Build history of the part. All positions in model axes, mm. A direction names the side the tool comes from. Round coordinates to 2 decimals unless told otherwise and drop trailing zeros. Loops run counter-clockwise (first coordinate to the right, second up) from the corner with the lowest first, then second, coordinate; pieces in that order, holes last. Notation, with made-up numbers: (48, -39) - (64, -39) arc R16 ccw to (64, -21) - close; hole circle Ø7 at (1, -0.75). An arc over 180 degrees is marked (long way). Use a Markdown table: item, result.
from build123d import *

# Parameters (mm, degrees)
SKETCH1_W                   = 85
SKETCH1_H                   = 80
BOSS_EXTRUDE1_DEPTH         = 40
M8_TAPPED_HOLE1_D           = 6.8
M8_TAPPED_HOLE1_DEPTH       = 22.25
M8_TAPPED_HOLE1_CSINK_D     = 8.05
M8_TAPPED_HOLE1_CSINK_ANGLE = 90
M8_TAPPED_HOLE1_TIP         = 2.042926105
SKETCH5_W                   = 20
SKETCH5_H                   = 54.3
CUT_EXTRUDE1_DEPTH          = 1
CUT_EXTRUDE2_DEPTH          = 12


with BuildPart() as part:
    # Sketch1 → Boss-Extrude1 (new body)
    with BuildSketch(Plane(origin=(0, 0, 0), x_dir=(1, 0, 0), z_dir=(0, 1, 0))):
        Rectangle(SKETCH1_W, SKETCH1_H)
    extrude(amount=BOSS_EXTRUDE1_DEPTH)

    # M8 Tapped Hole1
    with Locations(Plane(origin=(0, 0, 0), x_dir=(-1, 0, 0), z_dir=(0, -1, 0))):
        with Locations((7.5, 28), (-22.5, 0), (7.5, -28), (32.5, 0)):
            CounterSinkHole(M8_TAPPED_HOLE1_D / 2, M8_TAPPED_HOLE1_CSINK_D / 2, depth=M8_TAPPED_HOLE1_DEPTH, counter_sink_angle=M8_TAPPED_HOLE1_CSINK_ANGLE)
            with Locations((0, 0, -(M8_TAPPED_HOLE1_DEPTH + M8_TAPPED_HOLE1_TIP / 2))):  # 118° drill point
                Cone(0, M8_TAPPED_HOLE1_D / 2, M8_TAPPED_HOLE1_TIP, mode=Mode.SUBTRACT)

    # Sketch5 → Cut-Extrude1 (cut)
    with BuildSketch(Plane(origin=(0, 40, 0), x_dir=(1, 0, 0), z_dir=(0, 1, 0))):
        with Locations((-7.5, 0)):
            Rectangle(SKETCH5_W, SKETCH5_H)
    extrude(amount=-CUT_EXTRUDE1_DEPTH, mode=Mode.SUBTRACT)

    # Sketch6 → Cut-Extrude2 (cut, symmetric)
    with BuildSketch(Plane.ZY.offset(7.5)):
        with BuildLine():
            Line((-8.2, 40), (8.2, 40))
            ThreePointArc((8.2, 40), (6.414845549, 34.892186713), (1.836644737, 32.008333333))
            ThreePointArc((1.836644737, 32.008333333), (1.264123473, 32.045632996), (0.806331836, 32.391463415))
            ThreePointArc((0.806331836, 32.391463415), (0, 32.8), (-0.806331836, 32.391463415))
            ThreePointArc((-0.806331836, 32.391463415), (-1.264123473, 32.045632996), (-1.836644737, 32.008333333))
            ThreePointArc((-1.836644737, 32.008333333), (-6.414845549, 34.892186713), (-8.2, 40))
        make_face()
    extrude(amount=CUT_EXTRUDE2_DEPTH, both=True, mode=Mode.SUBTRACT)


solid = part.part
Q1. Probe line 1 (Z direction, x = -7.5, y = 16.75); line 2 (X direction, y = 7, z = 28); line 3 (Z direction, x = -32.5, y = 7). List the from-to ranges inside material, lowest first.
Results found:
| item | result |
|---|---|
| line 1 | z = -40 to -31.4, -24.6 to 24.6, 31.4 to 40 |
| line 2 | x = -42.5 to -10.9, -4.1 to 42.5 |
| line 3 | z = -40 to -3.4, 3.4 to 40 |
Q2. Which spindle directions (+Z, -Z, +X, -X, +Y, -Y) get a long thin tool onto all of the face, cutting with end or side? Do faces 1 (the face through (-29.36, 11.59, 1.3)), 2 (the face through (42.5, 20, 1)), 3 (the face through (-7.7, 35, 6.5)). Say none if no direction does.
Results found:
| item | result |
|---|---|
| face 1 | -Y |
| face 2 | +Z, -Z, +X, +Y, -Y |
| face 3 | +Y |
Q3. Cut at B-B, the plane y = 35. List the corners of the cut face in (x, z), plus the area to 3 significant figures.
Results found:
| item | result |
|---|---|
| outline | (-42.5, -40) - (42.5, -40) - (42.5, 40) - (-42.5, 40) - close; hole (-19.5, -6.5) - (4.5, -6.5) - (4.5, 6.5) - (-19.5, 6.5) - close |
| area | 6,490 mm2 |
Q4. Drop a flat-ended pin along its axis: pin 1 (6 mm diameter, centred on x = 22.5, z = 0, fed in from -Y). Give the stop position or say it passes through.
Results found:
| item | result |
|---|---|
| pin 1 | stops at y = 22.49 |
Q5. Cut at A-A, the plane y = 6.5. List the corners of the cut face in (x, z).
Results found:
| item | result |
|---|---|
| outline | (-42.5, -40) - (42.5, -40) - (42.5, 40) - (-42.5, 40) - close; hole circle Ø6.8 at (-32.5, 0); hole circle Ø6.8 at (-7.5, -28); hole circle Ø6.8 at (-7.5, 28); hole circle Ø6.8 at (22.5, 0) |
